```python
from build123d import *

# Parameters (mm, degrees)
C_FRAME_BODY_DEPTH  = 4
FRAME_RIM_DEPTH     = 10
SCREW_BOSS_DEPTH    = 25
SCREW_BORE_SKETCH_R = 6
SCREW_BORE_12_DEPTH = 43
EDGE_FILLETS_R2_R   = 2


with BuildPart() as part:
    # C-Frame Profile Sketch → C-Frame Body (new, symmetric)
    with BuildSketch(Plane(origin=(0, 0, 0), x_dir=(0, 0, -1), z_dir=(1, 0, 0))):
        with BuildLine():
            Line((0, 75), (0, 30))
            ThreePointArc((0, 30), (8.786796564, 8.786796564), (30, 0))
            Line((30, 0), (90, 0))
            ThreePointArc((90, 0), (111.213203436, 8.786796564), (120, 30))
            Line((120, 30), (120, 68))
            Line((120, 68), (100, 98))
            Line((100, 98), (95, 98))
            Line((95, 98), (95, 30))
            ThreePointArc((95, 30), (93.535533906, 26.464466094), (90, 25))
            Line((90, 25), (30, 25))
            ThreePointArc((30, 25), (26.464466094, 26.464466094), (25, 30))
            Line((25, 30), (25, 75))
            Line((25, 75), (0, 75))
        make_face()
    extrude(amount=C_FRAME_BODY_DEPTH, both=True)

    # Frame Rim Sketch → Frame Rim (add, symmetric)
    with BuildSketch(Plane(origin=(0, 0, 0), x_dir=(0, 0, -1), z_dir=(1, 0, 0))):
        with BuildLine():
            Line((25, 75), (20, 75))
            Line((20, 75), (20, 30))
            ThreePointArc((20, 30), (22.928932188, 22.928932188), (30, 20))
            Line((30, 20), (90, 20))
            ThreePointArc((90, 20), (97.071067812, 22.928932188), (100, 30))
            Line((100, 30), (100, 98))
            Line((100, 98), (95, 98))
            Line((95, 98), (95, 30))
            ThreePointArc((95, 30), (93.535533906, 26.464466094), (90, 25))
            Line((90, 25), (30, 25))
            ThreePointArc((30, 25), (26.464466094, 26.464466094), (25, 30))
            Line((25, 30), (25, 75))
        make_face()
    extrude(amount=FRAME_RIM_DEPTH, both=True)

    # Screw Boss Sketch → Screw Boss (add)
    with BuildSketch(Plane.XY):
        with BuildLine():
            Line((-10, 75), (10, 75))
            Line((10, 75), (10, 88))
            ThreePointArc((10, 88), (0, 98), (-10, 88))
            Line((-10, 88), (-10, 75))
        make_face()
    extrude(amount=-SCREW_BOSS_DEPTH)

    # Screw Bore Sketch → Screw Bore Ø12 (cut)
    with BuildSketch(Plane.XY):
        with Locations((0, 88)):
            Circle(SCREW_BORE_SKETCH_R)
    extrude(amount=-SCREW_BORE_12_DEPTH, mode=Mode.SUBTRACT)

    # Edge Fillets R2
    edge_fillets_r2_edges = [part.edges().sort_by_distance(p)[0] for p in [
        (7, 75, -20),
        (-7, 75, -20),
    ]]
    fillet(edge_fillets_r2_edges, radius=EDGE_FILLETS_R2_R)


solid = part.part
```
Verification items for the finished model (mm, model axes). A direction names the side the tool comes from. Give positions to 0.01 mm unless a question says otherwise; leave off trailing zeros. Loops run counter-clockwise (first coordinate to the right, second up) from the corner with the lowest first, then second, coordinate; pieces in that order, holes last.
1. Go/stop test with flat-tipped pins: pin 1 Ø6 at (x, z) = (1, -72.5) entering from +Y; pin 2 Ø5 at (x, z) = (5.5, -6) entering from -Y; pin 3 Ø6.5 at (x, z) = (7.5, -52) entering from -Y. Record where each tip stops, or that it passes through.
2. Mould release check, pull along Z, two halves, no side actions. Record for faces 1 (the cylindrical face through (0, 27, -94)), 2 (the flat face through (0, 25, -60)), 3 (the flat face through (7, 75, -9)), 4 (the cylindrical face through (-6.96, 22.85, -96.99)): released by +Z, released by -Z, zero draft, split by the parting line, or undercut.
3. Set-up check for faces 5 (the flat face through (7, 52, -20)), 6 (the flat face through (-7, 20, -60)), 7 (the flat face through (7, 20, -60)): record each of +Z, -Z, +X, -X, +Y, -Y from which the full face is reachable in a straight line by a thin tool's end or side.
4. Section check C-C, the plane y = 92.5. Enter the section's corners in (x, z), then the cut area to 3 significant figures.
5. Section check D-D, the plane x = 7.5. Enter the section's corners in (y, z).
6. Section check B-B, the plane y = 65. Enter the section's corners in (x, z).
7. Section check A-A, the plane x = 0. Enter the section's corners in (y, z), then the cut area to 3 significant figures.
8. Thickness scan on line 1 (Z direction, x = -7, y = 80); line 2 (Z direction, x = 2.5, y = 32.5); line 3 (Y direction, x = -6, z = -53.5). Record the ranges inside material, lowest first.
Geometry says:
1. pin 1: stops at y = 25
1. pin 2: stops at y = 9.6
1. pin 3: stops at y = 20
2. face 1: undercut
2. face 2: undercut
2. face 3: zero draft
2. face 4: released by -Z
3. face 5: +Z, +X, -Y
3. face 6: +Z, -Z, -X, -Y
3. face 7: +Z, -Z, +X, -Y
4. outline: (-10, -100) - (-4, -100) - (-4, -103.67) - (4, -103.67) - (4, -100) - (10, -100) - (10, -95) - (-10, -95) - close; (-8.93, -25) - (-3.97, -25) - (-3.97, 0) - (-8.93, 0) - close; (3.97, -25) - (8.93, -25) - (8.93, 0) - (3.97, 0) - close
4. area: 377 mm2
5. outline: (20, -90) arc R10 ccw to (30, -100) - (98, -100) - (98, -95) - (30, -95) arc R5 cw to (25, -90) - (25, -30) arc R5 cw to (30, -25) - (94.61, -25) - (94.61, 0) - (75, 0) - (75, -18) arc R2 cw to (73, -20) - (30, -20) arc R10 ccw to (20, -30) - close
6. outline: (-10, -100) - (-4, -100) - (-4, -120) - (4, -120) - (4, -100) - (10, -100) - (10, -95) - (-10, -95) - close; (-10, -25) - (10, -25) - (10, -20) - (4, -20) - (4, 0) - (-4, 0) - (-4, -20) - (-10, -20) - close
7. outline: (0, -90) arc R30 ccw to (30, -120) - (68, -120) - (98, -100) - (98, -95) - (30, -95) arc R5 cw to (25, -90) - (25, -30) arc R5 cw to (30, -25) - (82, -25) - (82, 0) - (30, 0) arc R30 ccw to (0, -30) - close; (94, -25) - (98, -25) - (98, 0) - (94, 0) - close
7. area: 5,670 mm2
8. line 1: z = -100 to -95, -25 to 0
8. line 2: z = -120 to -95, -25 to 0
8. line 3: y = 20 to 25
